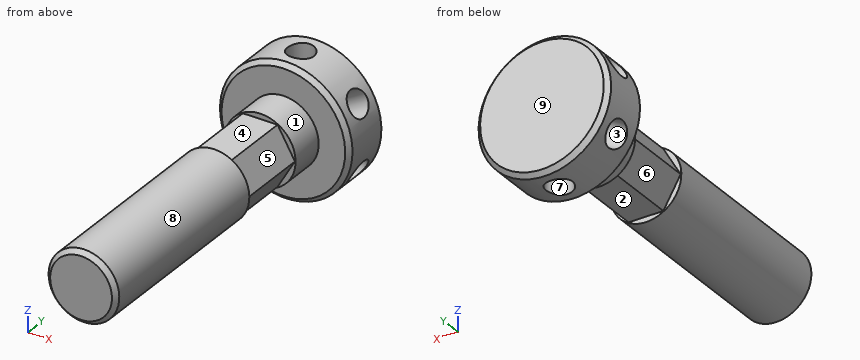
from build123d import *

# Parameters (mm, degrees)
SKETCH1_R           = 4
BOSS_EXTRUDE1_DEPTH = 35
SKETCH2_R           = 7.5
BOSS_EXTRUDE2_DEPTH = 6
CHAMFER1_SIZE       = 0.5
SKETCH3_R           = 1.5
CUT_EXTRUDE1_DEPTH  = 9.5
CIRPATTERN1_COUNT   = 6
SKETCH5_W           = 1.2
SKETCH5_H           = 8
CUT_EXTRUDE3_DEPTH  = 5
CIRPATTERN3_COUNT   = 6


with BuildPart() as part:
    # Sketch1 → Boss-Extrude1 (new body)
    with BuildSketch(Plane(origin=(0, 0, 0), x_dir=(1, 0, 0), z_dir=(0, 1, 0))):
        with Locations(Location((0, 0, 0), (0, 0, 270))):
            Circle(SKETCH1_R)
    extrude(amount=BOSS_EXTRUDE1_DEPTH)

    # Sketch2 → Boss-Extrude2 (add)
    with BuildSketch(Plane(origin=(0, 35, 0), x_dir=(1, 0, 0), z_dir=(0, 1, 0))):
        with Locations(Location((0, 0, 0), (0, 0, 270))):
            Circle(SKETCH2_R)
    extrude(amount=BOSS_EXTRUDE2_DEPTH)

    # Chamfer1
    chamfer1_edges = [part.edges().sort_by_distance(p)[0] for p in [
        (0, 0, -4),
        (0, 35, -7.5),
        (0, 41, -7.5),
    ]]
    chamfer(chamfer1_edges, length=CHAMFER1_SIZE)

    # Sketch3 → Cut-Extrude1 (cut, symmetric)
    with BuildSketch(Plane.XY):
        with Locations(Location((0, 38, 0), (0, 0, 90.000000044))):
            Circle(SKETCH3_R)
    cut_extrude1 = extrude(amount=CUT_EXTRUDE1_DEPTH, both=True, mode=Mode.SUBTRACT)

    # CirPattern1: Cut-Extrude1 ×6 about axis
    cirpattern1_axis = Axis((0, 41, 0), (0, -1, 0))
    for i in range(1, CIRPATTERN1_COUNT):
        add(cut_extrude1.rotate(cirpattern1_axis, i * 360 / CIRPATTERN1_COUNT), mode=Mode.SUBTRACT)

    # Sketch5 → Cut-Extrude3 (cut, symmetric)
    with BuildSketch(Plane(origin=(0, 0, 0), x_dir=(0, 0, -1), z_dir=(1, 0, 0))):
        with Locations((4, 27)):
            Rectangle(SKETCH5_W, SKETCH5_H)
    cut_extrude3 = extrude(amount=CUT_EXTRUDE3_DEPTH, both=True, mode=Mode.SUBTRACT)

    # CirPattern3: Cut-Extrude3 ×6 about axis
    cirpattern3_axis = Axis((0, 0, 0), (0, 1, 0))
    for i in range(1, CIRPATTERN3_COUNT):
        add(cut_extrude3.rotate(cirpattern3_axis, i * 360 / CIRPATTERN3_COUNT), mode=Mode.SUBTRACT)


solid = part.part
Read the model definition and answer for the solid it produces. Units are mm, in the model's axes. Face numbers are marked on the shaded views. A direction names the side the tool comes from. Give positions to 0.01 mm unless a question says otherwise; leave off trailing zeros. Loops run counter-clockwise (first coordinate to the right, second up) from the corner with the lowest first, then second, coordinate; pieces in that order, holes last. Notation, with made-up numbers: (16, 70.5) -> (74, 70.5) arc R17 ccw to (74, 98.5) -> close; hole circle Ø9 at (12.5, 16.5). An arc over 180 degrees is marked (long way). Answer as CSV lines item,"result".
Item 1: For the marked faces 1, 2, 3, 4 and 5, determine the directions among +Z, -Z, +X, -X, +Y, -Y from which every point of the face is accessible in a straight line to the end or side of a thin tool.
Returned:
face 1,"-Y"
face 2,"-Z, +X, -X"
face 3,"none"
face 4,"+Z, +X, -X"
face 5,"+Z, +X"
Item 2: Find section C-C on y = 9. Give the vertices of the cut face in (x, z), plus the area to 3 significant figures.
Returned:
outline,"circle Ø8 at (0, 0)"
area,"50.3 mm²"
Item 3: Determine the mould class of the marked faces 6, 7, 8 and 9 for opening direction X: +X half, -X half, draft (parallel to the pull), parting line (faces both ways), or undercut.
Returned:
face 6,"-X half"
face 7,"undercut"
face 8,"parting line"
face 9,"draft"
Item 4: Consider line 1 (Y direction, x = 0, z = 2.75); line 2 (Z direction, x = 5.25, y = 37.5); line 3 (X direction, y = 12, z = 0.25). Determine where each line is inside the solid, lowest interval first. Write a range as [from, to].
Returned:
line 1,"y = [0, 36.5], [39.5, 41]"
line 2,"z = [-5.36, -4.66], [-1.4, 1.4], [4.66, 5.36]"
line 3,"x = [-3.99, 3.99]"
Item 5: Find section B-B on y = 29. Give the vertices of the cut face in (x, z), plus the area to 3 significant figures.
Returned:
outline,"(-3.93, 0) -> (-1.96, -3.4) -> (1.96, -3.4) -> (3.93, 0) -> (1.96, 3.4) -> (-1.96, 3.4) -> close"
area,"40.0 mm²"
Item 6: Each of these flat-tipped pins is pushed along its axis until it touches: pin 1 (1.5 mm diameter, centred on x = 2.5, y = 18, fed in from +Z); pin 2 (2 mm diameter, centred on x = 4.5, z = -4.5, fed in from -Y); pin 3 (8 mm diameter, centred on y = 13.5, z = 4.5, fed in from +X); pin 4 (2.5 mm diameter, centred on x = 0, y = 38, fed in from -Z). Where does it stop, or does it pass through?
Returned:
pin 1,"stops at z = 3.6"
pin 2,"stops at y = 35"
pin 3,"stops at x = 3.97"
pin 4,"passes through"
Item 7: Find section A-A on y = 38. Give the vertices of the cut face in (x, z).
Returned:
outline,"(-7.11, -2.38) -> (-3, 0) -> (-7.11, 2.38) arc R7.5 ccw to start; (-5.61, -4.97) arc R7.5 ccw to (-1.5, -7.35) -> (-1.5, -2.6) -> close; (-5.61, 4.97) -> (-1.5, 2.6) -> (-1.5, 7.35) arc R7.5 ccw to start; (1.5, -7.35) arc R7.5 ccw to (5.61, -4.97) -> (1.5, -2.6) -> close; (1.5, 2.6) -> (5.61, 4.97) arc R7.5 ccw to (1.5, 7.35) -> close; (3, 0) -> (7.11, -2.38) arc R7.5 ccw to (7.11, 2.38) -> close"
